Check sheet for the modelled part. Datum: model origin and axes. Units: mm. Round coordinates to 2 decimals unless told otherwise and drop trailing zeros. Loops run counter-clockwise (first coordinate to the right, second up) from the corner with the lowest first, then second, coordinate; pieces in that order, holes last. Notation, with made-up numbers: (1, 89) - (31, 89) arc R21 cw to (31, 127) - close; hole circle Ø1 at (81, -17.5). An arc over 180 degrees is marked (long way). Put each result on its own line as item: value. Start each with the question number.
```python
from build123d import *

# Parameters (mm, degrees)
EXTRUDE_1_DEPTH = 7.5


with BuildPart() as part:
    # 草图2 → 拉伸-薄壁1 (new, symmetric)
    with BuildSketch(Plane.XY):
        with BuildLine():
            Line((20.415, 1455), (20.415, 0))
            ThreePointArc((20.415, 0), (0, -20.415), (-20.415, 0))
            Line((-20.415, 0), (-20.415, 1455))
            ThreePointArc((-20.415, 1455), (0, 1475.415), (20.415, 1455))
        make_face()
        with BuildLine():
            Line((19.415, 1455), (19.415, 0))
            ThreePointArc((19.415, 0), (0, -19.415), (-19.415, 0))
            Line((-19.415, 0), (-19.415, 1455))
            ThreePointArc((-19.415, 1455), (0, 1474.415), (19.415, 1455))
        make_face(mode=Mode.SUBTRACT)
    extrude(amount=EXTRUDE_1_DEPTH, both=True)


solid = part.part
```
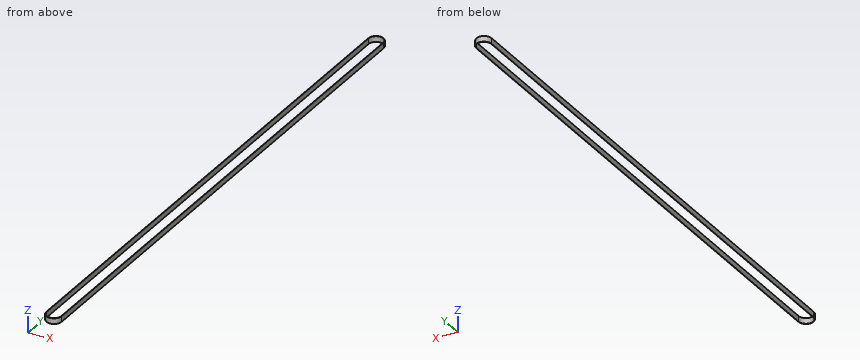
Q1. Cross-section at A-A on x = 0. Enter the section's corners in (y, z) (3 decimals).
Q2. Cross-section at C-C on z = -3. Enter the section's corners in (x, y) (3 decimals).
Q3. Material ranges on line 1 (Y direction, x = 2, z = -2.75); line 2 (X direction, y = 480, z = 1) (3 decimals); line 3 (Y direction, x = -3, z = -1.5), recorded low to high. Write a range as from..to.
Q4. Cross-section at B-B on y = 840. Enter the section's corners in (x, z) (3 decimals).
Q5. Depth check by flat-ended pin: pin 1 Ø8 at (x, z) = (-2, 4.5) entering from -Y (3 decimals). Enter the tip coordinate at first touch or a pass-through.
Answer list:
1. outline: (-20.415, -7.5) - (-19.415, -7.5) - (-19.415, 7.5) - (-20.415, 7.5) - close; (1474.415, -7.5) - (1475.415, -7.5) - (1475.415, 7.5) - (1474.415, 7.5) - close
2. outline: (-20.415, 0) arc R20.415 ccw to (20.415, 0) - (20.415, 1455) arc R20.415 ccw to (-20.415, 1455) - close; hole (-19.415, 0) arc R19.415 ccw to (19.415, 0) - (19.415, 1455) arc R19.415 ccw to (-19.415, 1455) - close
3. line 1: y = -20.32..-19.31, 1474.31..1475.32
3. line 2: x = -20.415..-19.415, 19.415..20.415
3. line 3: y = -20.19..-19.18, 1474.18..1475.19
4. outline: (-20.415, -7.5) - (-19.415, -7.5) - (-19.415, 7.5) - (-20.415, 7.5) - close; (19.415, -7.5) - (20.415, -7.5) - (20.415, 7.5) - (19.415, 7.5) - close
5. pin 1: stops at y = -20.415
